from build123d import *

# Parameters (mm, degrees)
SKETCH_1_R               = 12.5
EXTRUDE_1_DEPTH          = 315
SKETCH_2_R               = 10
EXTRUDE_2_DEPTH          = 30
EXTRUDE_START            = 20
SKETCH_3_R               = 10
EXTRUDE_3_DEPTH          = 20
CHAMFER_1_SIZE           = 0.5
SKETCH_4_R               = 7
EXTRUDE_4_DEPTH          = 40
CHAMFER_2_SIZE           = 0.5
CUT_EXTRUDE_1_DEPTH      = 376.416435442
CUT_EXTRUDE_1_DEPTH_BACK = 376.416435442
SKETCH_5_R               = 3
SKETCH_6_R               = 16.937839691
SKETCH_6_W               = 11.8
SKETCH_6_H               = 11.8
CUT_EXTRUDE_2_DEPTH      = 10


with BuildPart() as part:
    # 草图1 → 凸台-拉伸1 (new, symmetric)
    with BuildSketch(Plane.XY):
        Circle(SKETCH_1_R)
    extrude(amount=EXTRUDE_1_DEPTH, both=True)

    # 草图2 → 凸台-拉伸2 (add)
    with BuildSketch(Plane.XY.offset(315)):
        Circle(SKETCH_2_R)
    extrude(amount=EXTRUDE_2_DEPTH)

    # 草图3 → 凸台-拉伸3 (add)
    with BuildSketch(Plane(origin=(0, 0, -315), x_dir=(-1, 0, 0), z_dir=(0, 0, -1)).offset(EXTRUDE_START)):
        with Locations(Location((0, 0, 0), (0, 0, 180))):
            Circle(SKETCH_3_R)
    extrude(amount=-EXTRUDE_3_DEPTH)

    # 倒角1
    chamfer_1_edges = [part.edges().sort_by_distance(p)[0] for p in [
        (-10, 0, -335),
        (-10, 0, 345),
    ]]
    chamfer(chamfer_1_edges, length=CHAMFER_1_SIZE)

    # 草图4 → 凸台-拉伸4 (add)
    with BuildSketch(Plane(origin=(0, 0, -335), x_dir=(-1, 0, 0), z_dir=(0, 0, -1))):
        Circle(SKETCH_4_R)
    extrude(amount=EXTRUDE_4_DEPTH)

    # 倒角2
    chamfer_2_edges = [part.edges().sort_by_distance(p)[0] for p in [
        (7, 0, -375),
    ]]
    chamfer(chamfer_2_edges, length=CHAMFER_2_SIZE)

    # 草图5 → 切除-拉伸1 (cut, two sides: drawn at the far end of the back side and taken through both)
    with BuildSketch(Plane(origin=(0, 0, 0), x_dir=(0, 0, -1), z_dir=(1, 0, 0)).offset(-CUT_EXTRUDE_1_DEPTH_BACK)):
        with Locations((367, 0)):
            Circle(SKETCH_5_R)
    extrude(amount=CUT_EXTRUDE_1_DEPTH + CUT_EXTRUDE_1_DEPTH_BACK, mode=Mode.SUBTRACT)

    # 草图6 → 切除-拉伸2 (cut)
    with BuildSketch(Plane.XY.offset(345)):
        Circle(SKETCH_6_R)
        Rectangle(SKETCH_6_W, SKETCH_6_H, mode=Mode.SUBTRACT)
    extrude(amount=-CUT_EXTRUDE_2_DEPTH, mode=Mode.SUBTRACT)


solid = part.part
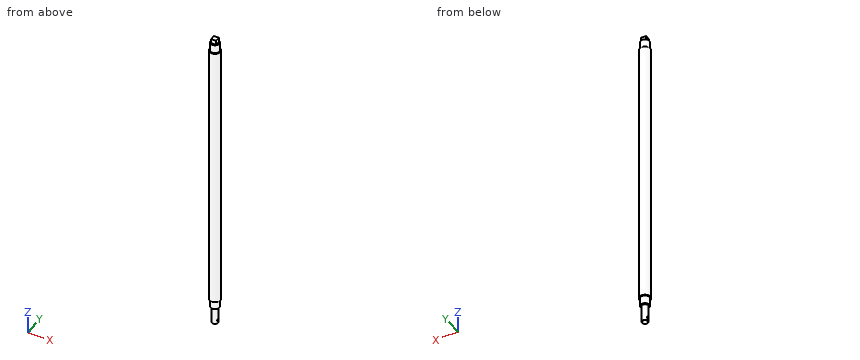
Part model, mm, in its own coordinate system. Coordinates: 2 decimals unless noted, no trailing zeros. Loops run counter-clockwise (first coordinate to the right, second up) from the corner with the lowest first, then second, coordinate; pieces in that order, holes last. Notation, with made-up numbers: (62, 5.5) -> (93, 5.5) arc R24 ccw to (93, 33.5) -> close; hole circle Ø10 at (-7, -23.5). An arc over 180 degrees is marked (long way). Use a Markdown table: item, result. Add a question column.
Item 1: Probe probe 1 along Z at (x, y) = (1, 0); probe 2 along Y at (x, z) = (-2.5, -367); probe 3 along Z at (x, y) = (-10.5, 3.75). List the from-to ranges inside material, lowest first.
Item 2: Band-saw the part on B-B on z = -308.5. Write the cut outline in (x, y).
Item 3: Band-saw the part on A-A on x = 0. Write the cut outline in (y, z).
Item 4: Flat gauge pins, fed straight in: P1, Ø4, axis at x = -6, z = -273, coming from the +Y side; P2, Ø11, axis at y = -1.5, z = 342, coming from the +X side; P3, Ø8, axis at x = -6, y = -9.5, coming from the -Z side. Where does each tip first touch, or does it go through?
Geometry says:
| question | item | result |
|---|---|---|
| 1 | probe 1 | -375 to -370, -364 to 345 |
| 1 | probe 2 | -6.54 to -3, 3 to 6.54 |
| 1 | probe 3 | -315 to 315 |
| 2 | outline | circle Ø25 at (0, 0) |
| 3 | outline | (-12.5, -315) -> (-10, -315) -> (-10, -334.5) -> (-9.5, -335) -> (-7, -335) -> (-7, -374.5) -> (-6.5, -375) -> (6.5, -375) -> (7, -374.5) -> (7, -335) -> (9.5, -335) -> (10, -334.5) -> (10, -315) -> (12.5, -315) -> (12.5, 315) -> (10, 315) -> (10, 335) -> (5.9, 335) -> (5.9, 345) -> (-5.9, 345) -> (-5.9, 335) -> (-10, 335) -> (-10, 315) -> (-12.5, 315) -> close; hole circle Ø6 at (0, -367) |
| 4 | P1 | y = 11.84 |
| 4 | P2 | x = 5.9 |
| 4 | P3 | z = -335 |
